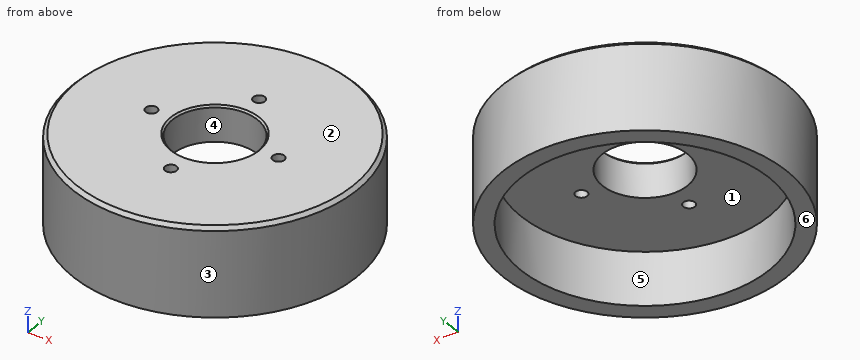
```python
from build123d import *

# Parameters (mm, degrees)
CHAMFER1_SIZE      = 1
SKETCH9_R          = 12
CUT_EXTRUDE1_DEPTH = 62.846584384
M4_TAPPED_HOLE1_D  = 3.3
CHAMFER2_SIZE      = 0.5


with BuildPart() as part:
    # Sketch8 → Revolve2 (revolve)
    with BuildSketch(Plane(origin=(0, 0, 0), x_dir=(0, 0, -1), z_dir=(1, 0, 0)), mode=Mode.PRIVATE) as revolve2_sk:
        Polygon((0, 0), (0, 40), (25, 40), (25, 35), (10, 35), (10, 0), align=None)
    revolve(revolve2_sk.sketch.rotate(Axis((0, 0, 0), (0, 0, -1)), 90), axis=Axis((0, 0, 0), (0, 0, -1)))

    # Chamfer1
    chamfer1_edges = [part.edges().sort_by_distance(p)[0] for p in [
        (-40, 0, 0),
    ]]
    chamfer(chamfer1_edges, length=CHAMFER1_SIZE)

    # Sketch9 → Cut-Extrude1 (cut, through all)
    with BuildSketch(Plane.XY):
        Circle(SKETCH9_R)
    extrude(amount=-CUT_EXTRUDE1_DEPTH, mode=Mode.SUBTRACT)

    # M4 Tapped Hole1 (through all)
    with Locations(Plane(origin=(0, 18, 0), x_dir=(1, 0, 0), z_dir=(0, 0, 1))):
        with Locations((0, 0), (-18, -18), (18, -18), (0, -36)):
            Hole(M4_TAPPED_HOLE1_D / 2)

    # Chamfer2
    chamfer2_edges = [part.edges().sort_by_distance(p)[0] for p in [
        (-12, 0, 0),
    ]]
    chamfer(chamfer2_edges, length=CHAMFER2_SIZE)


solid = part.part
```
CAD build for the part. Positions are in the model's coordinates, mm. Face numbers are marked on the shaded views. A direction names the side the tool comes from. Round coordinates to 2 decimals unless told otherwise and drop trailing zeros. Loops run counter-clockwise (first coordinate to the right, second up) from the corner with the lowest first, then second, coordinate; pieces in that order, holes last. Notation, with made-up numbers: M -24.75,2 L 33.25,2 A15 cw 33.25,17 Z; hole C 42,11 d1. An arc over 180 degrees is marked long. Return JSON: item names as keys, results as strings. Group by question number.
(1) Drop flat-ended pins along their axis: P1, Ø3, axis at y = 23, z = -5.5, coming from the -X side; P2, Ø8, axis at x = -7, z = -10.5, coming from the -Y side; P3, Ø3, axis at x = 18, y = 0, coming from the -Z side; P4, Ø1, axis at x = 29, z = -9.5, coming from the +Y side. Give the stop position or say it passes through.
(2) Tool access for the marked faces 5 and 6: list every direction of +Z, -Z, +X, -X, +Y, -Y with a clear straight run to the whole face (end or side of a thin tool).
(3) Saw through at C-C, the plane z = -18. List the corners of the cut face in (x, y).
(4) Saw through at A-A, the plane y = 0. List the corners of the cut face in (x, z), and give its area (3 significant figures).
(5) Mould opens along X. For the marked faces 1, 2, 3 and 4 say: +X half, -X half, draft (parallel to the pull), parting line (faces both ways), or undercut.
(6) Wall check: probe 1 along Y at (x, z) = (0, -3.5); probe 2 along Y at (x, z) = (0, -13.5); probe 3 along Z at (x, y) = (14.5, 21). Give the ranges that are in metal, low to high. Write a range as [from, to].
Answer list:
{
 "1": {"P1": "x = -33.73", "P2": "y = -39.89", "P3": "through", "P4": "y = 28.07"},
 "2": {"face 5": "-Z", "face 6": "-Z, +X, -X, +Y, -Y"},
 "3": {"outline": "C 0,0 d80; hole C 0,0 d70"},
 "4": {"outline": "M -40,-25 L -35,-25 L -35,-10 L -19.65,-10 L -19.65,0 L -39,0 L -40,-1 Z; M -16.35,-10 L -12,-10 L -12,-0.5 L -12.5,0 L -16.35,0 Z; M 12,-10 L 16.35,-10 L 16.35,0 L 12.5,0 L 12,-0.5 Z; M 19.65,-10 L 35,-10 L 35,-25 L 40,-25 L 40,-1 L 39,0 L 19.65,0 Z", "area": "643 mm2"},
 "5": {"face 1": "undercut", "face 2": "draft", "face 3": "parting line", "face 4": "undercut"},
 "6": {"probe 1": "[-40, -19.65], [-16.35, -12], [12, 16.35], [19.65, 40]", "probe 2": "[-40, -35], [35, 40]", "probe 3": "[-10, 0]"}
}
